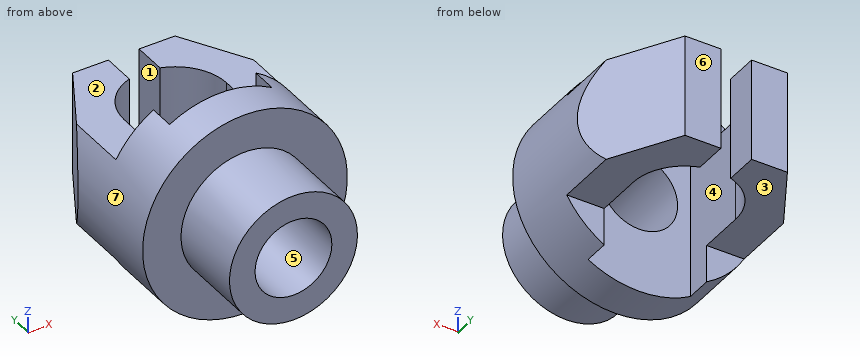
from build123d import *

# Parameters (mm, degrees)
FORK_SIDE_PROFILE_CUT_DEPTH      = 120.268604419
FORK_SIDE_PROFILE_CUT_DEPTH_BACK = 120.268604419
FORK_SIDE_PROFILE_SKETCH_W       = 20
FORK_SIDE_PROFILE_SKETCH_H       = 50
FORK_SLOT_CUT_DEPTH              = 120.268604419
FORK_SLOT_CUT_DEPTH_BACK         = 120.268604419


with BuildPart() as part:
    # Body Profile Sketch → Revolved Body (revolve)
    with BuildSketch(Plane.XY, mode=Mode.PRIVATE) as revolved_body_sk:
        Polygon((15, 0), (25, 0), (25, 30), (40, 30), (40, 105), (0, 105), (0, 55), (15, 55), align=None)
    revolve(revolved_body_sk.sketch.rotate(Axis((0, 0, 0), (0, 1, 0)), 90), axis=Axis((0, 0, 0), (0, 1, 0)))

    # Fork Side Profile Sketch → Fork Side Profile Cut (cut, two sides: drawn at the far end of the back side and taken through both)
    with BuildSketch(Plane(origin=(0, 0, 0), x_dir=(0, 0, -1), z_dir=(1, 0, 0)).offset(-FORK_SIDE_PROFILE_CUT_DEPTH_BACK)):
        with Locations((-30, 80)):
            Rectangle(FORK_SIDE_PROFILE_SKETCH_W, FORK_SIDE_PROFILE_SKETCH_H)
        with Locations((30, 80)):
            Rectangle(FORK_SIDE_PROFILE_SKETCH_W, FORK_SIDE_PROFILE_SKETCH_H)
    extrude(amount=FORK_SIDE_PROFILE_CUT_DEPTH + FORK_SIDE_PROFILE_CUT_DEPTH_BACK, mode=Mode.SUBTRACT)

    # Fork Slot Sketch → Fork Slot Cut (cut, two sides: drawn at the far end of the back side and taken through both)
    with BuildSketch(Plane.XY.offset(-FORK_SLOT_CUT_DEPTH_BACK)):
        Polygon((-40, 105), (-20, 105), (-40, 70), align=None)
        Polygon((40, 105), (20, 105), (40, 70), align=None)
        with BuildLine():
            Line((-20, 45), (20, 45))
            Line((20, 45), (20, 73))
            ThreePointArc((20, 73), (16.124515497, 84.832159566), (6, 92.078784028))
            Line((6, 92.078784028), (6, 105))
            Line((6, 105), (-6, 105))
            Line((-6, 105), (-6, 92.078784028))
            ThreePointArc((-6, 92.078784028), (-16.124515497, 84.832159566), (-20, 73))
            Line((-20, 73), (-20, 45))
        make_face()
    extrude(amount=FORK_SLOT_CUT_DEPTH + FORK_SLOT_CUT_DEPTH_BACK, mode=Mode.SUBTRACT)


solid = part.part
The model under review builds one solid part; all positions refer to its coordinate system, in mm. Face numbers are marked on the shaded views. A direction names the side the tool comes from. Give positions to 0.01 mm unless a question says otherwise; leave off trailing zeros. Write each loop counter-clockwise with the first axis right and the second up, starting at its lowest first coordinate (ties: lowest second). Pieces come first, ordered by that corner, then holes. Notation, with made-up numbers: M 38.25,50.5 L 94.25,50.5 A25 cw 94.25,76.5 Z; hole C 22.5,-32.5 d6. An arc over 180 degrees is marked long. One line per question, with ' | ' between items. Start each with the question number.
Item 1: We need section B-B on x = 13.5. Write out the cut boundary in (y, z), plus the area to 3 significant figures.
Item 2: Wall thickness on line 1 (X direction, y = 29.5, z = 0); line 2 (X direction, y = 67.5, z = 1); line 3 (Y direction, x = 19.5, z = 22): over which ranges is each line inside the solid? List them lowest first. Write a range as from..to.
Item 3: Draft analysis for pull direction X (two halves, no side actions). For the marked faces 5, 6 and 7, state which applies: released by +X, released by -X, zero draft, split by the parting line, or undercut.
Item 4: We need section A-A on z = 0. Write out the cut boundary in (x, y).
Item 5: For pin 1 (14 mm diameter, centred on y = 100.5, z = -4, fed in from +X); pin 2 (12 mm diameter, centred on x = -18, y = 64.5, fed in from -Z); pin 3 (2 mm diameter, centred on x = -1, z = 25, fed in from -Y); pin 4 (5 mm diameter, centred on x = -9, z = 5.5, fed in from -Y), all flat-tipped, find the tip position at first contact; note any pin that passes through.
Item 6: For the marked faces 1, 2, 3 and 4, list the 3-axis set-ups (+Z, -Z, +X, -X, +Y, -Y) from which the entire face can be reached by the end or side of a thin tool; tool diameter is ignored.
Item 7: We need section D-D on y = 49. Write out the cut boundary in (x, z).
Item 8: We need section C-C on x = 0. Write out the cut boundary in (y, z), plus the area to 3 significant figures.
Results found:
1) outline: M 0,-21.04 L 30,-21.04 L 30,-37.65 L 45,-37.65 L 45,-6.54 L 0,-6.54 Z; M 0,6.54 L 45,6.54 L 45,37.65 L 30,37.65 L 30,21.04 L 0,21.04 Z; M 87.76,-20 L 105,-20 L 105,20 L 87.76,20 Z | area: 2,490 mm2
2) line 1: x = -25..-15, 15..25 | line 2: x = -39.99..-20, 20..39.99 | line 3: y = 30..45
3) face 5: undercut | face 6: zero draft | face 7: split by the parting line
4) outline: M -40,30 L -25,30 L -25,0 L -15,0 L -15,45 L -20,45 L -20,73 A20 cw -6,92.08 L -6,105 L -20,105 L -40,70 Z; M 6,92.08 A20 cw 20,73 L 20,45 L 15,45 L 15,0 L 25,0 L 25,30 L 40,30 L 40,70 L 20,105 L 6,105 Z
5) pin 1: stops at x = 26.57 | pin 2: stops at z = -20 | pin 3: stops at y = 0 | pin 4: stops at y = 89.36
6) face 1: +Z, -Z, +Y | face 2: +Z, +X, -X, +Y | face 3: -Z, +X, -X, +Y | face 4: +Z, -Z
7) outline: M -20,-34.64 L -20,34.64 A40 ccw Z; M 20,-34.64 A40 ccw 20,34.64 Z
8) outline: M 0,-25 L 30,-25 L 30,-40 L 45,-40 L 45,-15 L 0,-15 Z; M 0,15 L 45,15 L 45,40 L 30,40 L 30,25 L 0,25 Z | area: 1,350 mm2
